```python
from build123d import *

# Parameters (mm, degrees)
SKETCH_1_W                  = 67
SKETCH_1_H                  = 46.3
EXTRUDE_1_DEPTH             = 2
FILLET_1_R                  = 6
HOLE_WIZARD_1_D             = 3.5
HOLE_WIZARD_1_DEPTH         = 10
HOLE_WIZARD_1_CSINK_D       = 6.5
HOLE_WIZARD_1_CSINK_ANGLE   = 90
PATTERN_LINEAR_1_COUNT      = 2
PATTERN_LINEAR_1_PITCH      = 34
PATTERN_LINEAR_1_COUNT_DIR2 = 2
PATTERN_LINEAR_1_PITCH_DIR2 = 59


with BuildPart() as part:
    # 草图1 → 拉伸1 (new body)
    with BuildSketch(Plane.XY):
        Rectangle(SKETCH_1_W, SKETCH_1_H)
    extrude(amount=EXTRUDE_1_DEPTH)

    # 圆角1
    fillet_1_edges = [part.edges().sort_by_distance(p)[0] for p in [
        (-33.5, 23.15, 1),
        (33.5, 23.15, 1),
        (33.5, -23.15, 1),
        (-33.5, -23.15, 1),
    ]]
    fillet(fillet_1_edges, radius=FILLET_1_R)

    # 孔1
    with Locations(Plane(origin=(-29.5, -17, 2), x_dir=(1, 0, 0), z_dir=(0, 0, 1))):
        with Locations((0, 0)):
            hole_wizard_1 = CounterSinkHole(HOLE_WIZARD_1_D / 2, HOLE_WIZARD_1_CSINK_D / 2, depth=HOLE_WIZARD_1_DEPTH, counter_sink_angle=HOLE_WIZARD_1_CSINK_ANGLE)

    # 阵列(线性)1: Hole Wizard 1 2 × 2
    with Locations(*[(j * PATTERN_LINEAR_1_PITCH_DIR2, i * PATTERN_LINEAR_1_PITCH, 0) for i in range(PATTERN_LINEAR_1_COUNT) for j in range(PATTERN_LINEAR_1_COUNT_DIR2) if (i, j) != (0, 0)]):
        add(hole_wizard_1, mode=Mode.SUBTRACT)


solid = part.part
```
Could you check a few things on this model? Use its own coordinates, in mm. Round coordinates to 2 decimals unless told otherwise and drop trailing zeros. Loops run counter-clockwise (first coordinate to the right, second up) from the corner with the lowest first, then second, coordinate; pieces in that order, holes last. Notation, with made-up numbers: M -13,44 L 3,44 A19 ccw 3,79 Z; hole C 49.5,-14.75 d7. An arc over 180 degrees is marked long. Put each result on its own line as item: value.
Q1. Imagine slicing it at B-B (x = 29.5). Write out the boundary of the cut face in (y, z).
Check result:
outline: M -22.81,0 L -18.75,0 L -18.75,0.5 L -20.25,2 L -22.81,2 Z; M -15.25,0 L 15.25,0 L 15.25,0.5 L 13.75,2 L -13.75,2 L -15.25,0.5 Z; M 18.75,0 L 22.81,0 L 22.81,2 L 20.25,2 L 18.75,0.5 Z
Q2. Imagine slicing it at C-C (y = 16). State how many separate pieces and enclosed holes the cut face has, then the cut area to 3 significant figures.
Check result:
separate pieces: 3
enclosed holes: 0
area: 117 mm2
Q3. I need wall thicknesses on probe 1 along X at (y, z) = (-17, 0.35); probe 2 along Y at (x, z) = (-29.5, 0.2); probe 3 along X at (y, z) = (-17, 1.4). Which ranges of each line are inside material? Lowest first, please.
Check result:
probe 1: -33.5 to -31.25, -27.75 to 27.75, 31.25 to 33.5
probe 2: -22.81 to -18.75, -15.25 to 15.25, 18.75 to 22.81
probe 3: -33.5 to -32.15, -26.85 to 26.85, 32.15 to 33.5
Q4. Thinking about a two-plate mould opening in X: for faces 1 (the face through (-33.5, 0, 1)), 2 (the face through (0, 0, 2)), 3 (the face through (-28.21, 18.18, 0.25)), which applies, released by +X, released by -X, zero draft, split by the parting line, or undercut?
Check result:
face 1: released by -X
face 2: zero draft
face 3: undercut
Q5. Imagine slicing it at A-A (z = 1.2). Write out the boundary of the cut face in (x, y), then the cut area to 3 significant figures.
Check result:
outline: M -33.5,-17.15 A6 ccw -27.5,-23.15 L 27.5,-23.15 A6 ccw 33.5,-17.15 L 33.5,17.15 A6 ccw 27.5,23.15 L -27.5,23.15 A6 ccw -33.5,17.15 Z; hole C -29.5,-17 d4.9; hole C -29.5,17 d4.9; hole C 29.5,-17 d4.9; hole C 29.5,17 d4.9
area: 3,000 mm2
Q6. For pin 1 (5.5 mm diameter, centred on x = -29.5, y = -17, fed in from -Z); pin 2 (2 mm diameter, centred on x = 29.5, y = -17, fed in from +Z); pin 3 (4 mm diameter, centred on x = -29.5, y = 17, fed in from +Z), each with a flat end and sliding along its axis, tell me the tip position at first contact or that it passes through.
Check result:
pin 1: z = 0
pin 2: through
pin 3: z = 0.75
